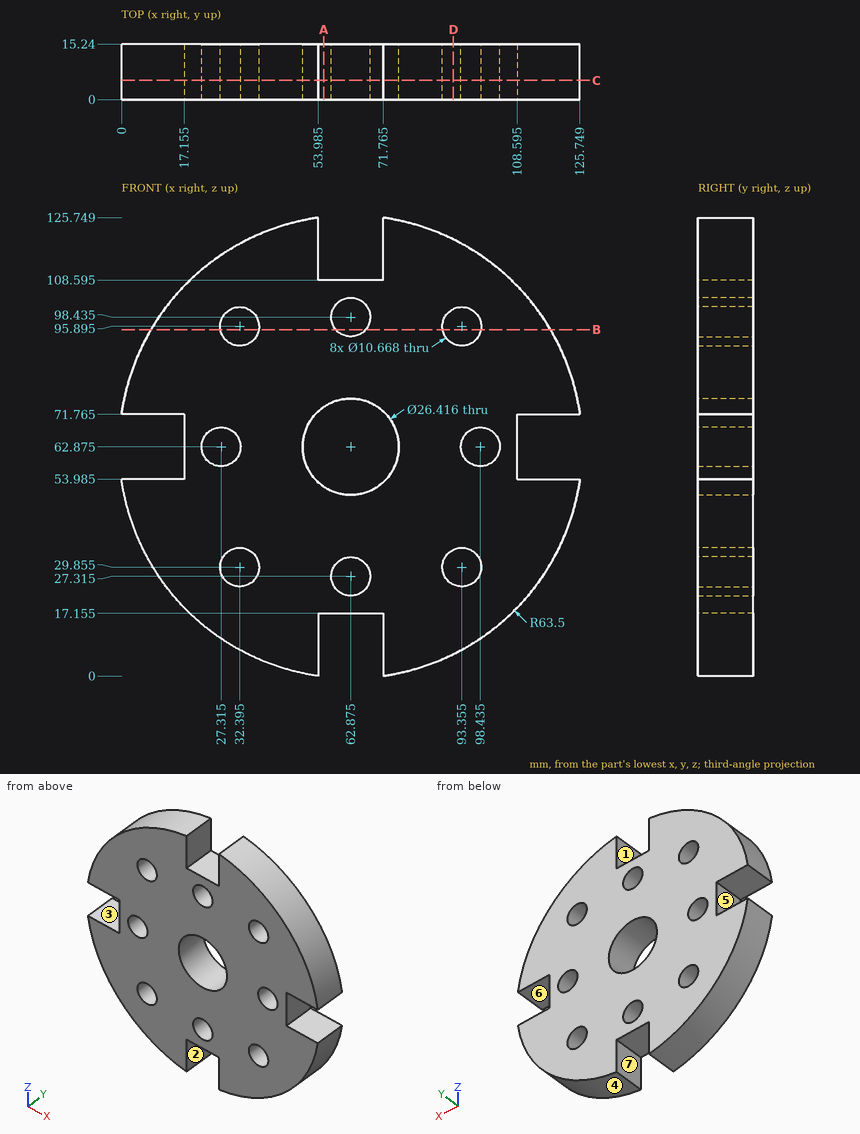
Verification items for this drawing (mm, ordinates from the low corner). A direction names the side the tool comes from. Round coordinates to 2 decimals unless told otherwise and drop trailing zeros. Write each loop counter-clockwise with the first axis right and the second up, starting at its lowest first coordinate (ties: lowest second). Pieces come first, ordered by that corner, then holes. Notation, with made-up numbers: (9, 18.25) - (26, 18.25) arc R17 cw to (26, 49.25) - close; hole circle Ø6 at (87.25, 37.25). An arc over 180 degrees is marked (long way). Answer as a JSON object with one key per item and string values. Group by question number.
Q1. Go/stop test with flat-tipped pins: pin 1 Ø4.5 at (y, z) = (8.5, 60.5) entering from +X (1 decimal); pin 2 Ø6 at (y, z) = (4.5, 22) entering from +X; pin 3 Ø4 at (x, y) = (99.5, 13.5) entering from +Z. Record where each tip stops, or that it passes through.
Q2. Section check B-B, the plane z = 95. Enter the section's corners in (x, y) (1 decimal).
Q3. Mould release check, pull along X, two halves, no side actions. Record for the marked faces 4, 5, 6 and 7: released by +X, released by -X, zero draft, split by the parting line, or undercut.
Q4. Section check C-C, the plane y = 5.25. Give the number of separate pieces and of enclosed holes in the cut face, plus the area to 3 significant figures.
Q5. Thickness scan on line 1 (Z direction, x = 65.5, y = 1) (1 decimal); line 2 (Z direction, x = 71.5, y = 13.5) (1 decimal); line 3 (X direction, y = 5.25, z = 93) (1 decimal). Record the ranges inside material, lowest first.
Q6. Section check A-A, the plane x = 55.5. Enter the section's corners in (y, z) (1 decimal).
Q7. Tool access check on the marked faces 1, 2 and 3. Record the directions out of +Z, -Z, +X, -X, +Y, -Y that give a thin tool (end or side, any length) a straight path to the whole face; none if there is none.
Q8. Section check D-D, the plane x = 91. Enter the section's corners in (y, z), plus the area to 3 significant figures.
Found:
{
 "1": {"pin 1": "stops at x = 108.6", "pin 2": "stops at x = 113.84", "pin 3": "stops at z = 116.1"},
 "2": {"outline": "(8.1, 0) - (27.1, 0) - (27.1, 15.2) - (8.1, 15.2) - close; (37.7, 0) - (58.8, 0) - (58.8, 15.2) - (37.7, 15.2) - close; (67, 0) - (88.1, 0) - (88.1, 15.2) - (67, 15.2) - close; (98.6, 0) - (117.6, 0) - (117.6, 15.2) - (98.6, 15.2) - close"},
 "3": {"face 4": "released by +X", "face 5": "released by -X", "face 6": "zero draft", "face 7": "undercut"},
 "4": {"separate pieces": "1", "enclosed holes": "9", "area": "10,200 mm^2"},
 "5": {"line 1": "z = 17.2 to 22.7, 32 to 49.9, 75.8 to 93.8, 103.1 to 108.6", "line 2": "z = 17.2 to 52.9, 72.9 to 108.6", "line 3": "x = 7 to 27.9, 36.9 to 88.9, 97.8 to 118.8"},
 "6": {"outline": "(0, 17.2) - (15.2, 17.2) - (15.2, 51.9) - (0, 51.9) - close; (0, 73.8) - (15.2, 73.8) - (15.2, 108.6) - (0, 108.6) - close"},
 "7": {"face 1": "+Z, +Y, -Y", "face 2": "-Z, +Y, -Y", "face 3": "-X, +Y, -Y"},
 "8": {"outline": "(0, 5.94) - (15.24, 5.94) - (15.24, 25.07) - (0, 25.07) - close; (0, 34.64) - (15.24, 34.64) - (15.24, 91.11) - (0, 91.11) - close; (0, 100.68) - (15.24, 100.68) - (15.24, 119.81) - (0, 119.81) - close", "area": "1,440 mm^2"}
}
